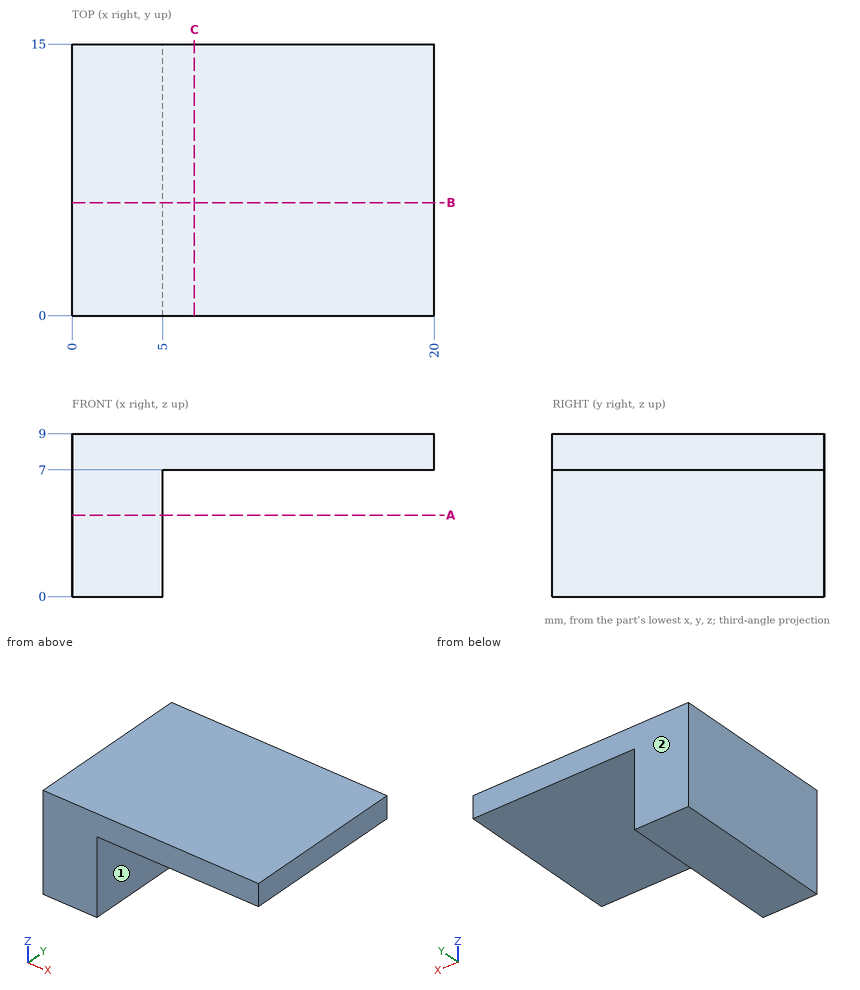
Could you check a few things on this drawing? It's one solid part, dimensions in mm from its lowest x, y, z. A direction names the side the tool comes from. Round coordinates to 2 decimals unless told otherwise and drop trailing zeros. Loops run counter-clockwise (first coordinate to the right, second up) from the corner with the lowest first, then second, coordinate; pieces in that order, holes last. Notation, with made-up numbers: (67.25, 37) -> (107.25, 37) arc R8 cw to (107.25, 45) -> close; hole circle Ø9 at (64, 61.5). An arc over 180 degrees is marked (long way). One line per item, written item: value. Start each with the question number.
1. If we section it at B-B, the plane y = 6.25: Write out the boundary of the cut face in (x, z), then the cut area to 3 significant figures.
2. For the marked faces 1 and 2, which set-ups out of +Z, -Z, +X, -X, +Y, -Y let a thin tool reach every point of the face, with its end or its side?
3. If I drill on probe 1 along Z at (x, y) = (18.25, 5.75); probe 2 along X at (y, z) = (8, 1.25), over which ranges is the centre line in solid material (lowest first)?
4. If we section it at A-A, the plane z = 4.5: Write out the boundary of the cut face in (x, y), then the cut area to 3 significant figures.
5. If we section it at C-C, the plane x = 6.75: Write out the boundary of the cut face in (y, z).
6. For pin 1 (2 mm diameter, centred on y = 8, z = 2.5, fed in from +X); pin 2 (3 mm diameter, centred on x = 13.5, y = 4, fed in from -Z), each with a flat end and sliding along its axis, tell me the tip position at first contact or that it passes through.
Calculated:
1. outline: (0, 0) -> (5, 0) -> (5, 7) -> (20, 7) -> (20, 9) -> (0, 9) -> close
1. area: 75.0 mm²
2. face 1: -Z, +X, +Y, -Y
2. face 2: +Z, -Z, +X, -X, +Y
3. probe 1: z = 7 to 9
3. probe 2: x = 0 to 5
4. outline: (0, 0) -> (5, 0) -> (5, 15) -> (0, 15) -> close
4. area: 75.0 mm²
5. outline: (0, 7) -> (15, 7) -> (15, 9) -> (0, 9) -> close
6. pin 1: stops at x = 5
6. pin 2: stops at z = 7
